Could you check a few things on this drawing? It's one solid part, dimensions in mm from its lowest x, y, z. A direction names the side the tool comes from. Give positions to 0.01 mm unless a question says otherwise; leave off trailing zeros. Loops run counter-clockwise (first coordinate to the right, second up) from the corner with the lowest first, then second, coordinate; pieces in that order, holes last. Notation, with made-up numbers: M 73.25,-15 L 101.25,-15 A24 ccw 101.25,-5 Z; hole C 29,65.5 d11. An arc over 180 degrees is marked long. Answer in a Markdown table with one row per item. Add a question column.
1. Which directions (+Z, -Z, +X, -X, +Y, -Y) give clear straight access to the entire face, cutting with the end or side of a thin tool? Please do the marked faces 1 and 2.
2. If we section it at D-D on x = 6: List the corners of the cut face in (y, z) for me, then the cut area to 3 significant figures.
3. Thinking about a two-plate mould opening in X: for the marked faces 3, 4, 5 and 6, which applies, released by +X, released by -X, zero draft, split by the parting line, or undercut?
4. If we section it at C-C on z = 3: List the corners of the cut face in (x, y) for me.
5. I need wall thicknesses on line 1 along Y through (x, z) = (34, 1.7); line 2 along Y through (x, z) = (34, 3.3); line 3 along X through (y, z) = (6.75, 5). Which ranges of each line are inside material? Lowest first, please. Write a range as from..to.
6. If we section it at B-B on y = 5: List the corners of the cut face in (x, z) for me.
7. I'm going to push flat-ended pins straight in: pin 1 Ø1.8 at (x, z) = (20.5, 4) entering from -Y; pin 2 Ø2.5 at (x, y) = (6, 5) entering from -Z; pin 3 Ø1.8 at (x, y) = (7, 6) entering from +Z; pin 4 Ø1.5 at (x, z) = (26, 3) entering from +Y. Where does each tip first touch, or does it pass through?
8. If we section it at A-A on x = 14: List the corners of the cut face in (y, z) for me.
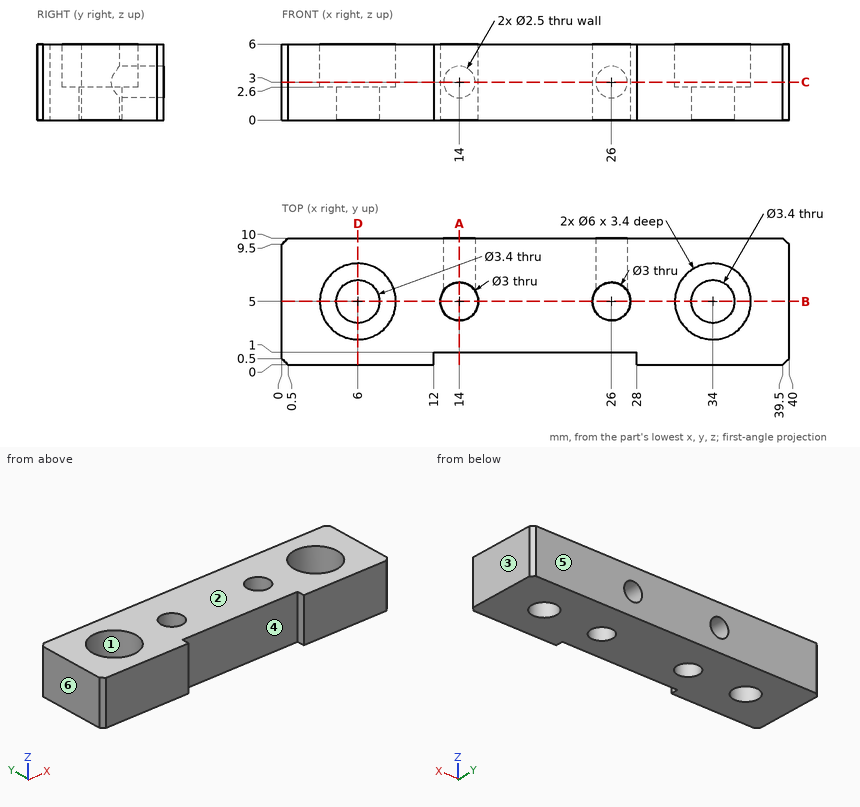
Results:
| question | item | result |
|---|---|---|
| 1 | face 1 | +Z |
| 1 | face 2 | +Z, +X, -X, +Y, -Y |
| 2 | outline | M 0,0 L 3.3,0 L 3.3,2.6 L 2,2.6 L 2,6 L 0,6 Z; M 6.7,0 L 10,0 L 10,6 L 8,6 L 8,2.6 L 6.7,2.6 Z |
| 2 | area | 30.8 mm2 |
| 3 | face 3 | released by +X |
| 3 | face 4 | undercut |
| 3 | face 5 | zero draft |
| 3 | face 6 | released by -X |
| 4 | outline | M 0,0.5 L 0.5,0 L 12,0 L 12,1 L 28,1 L 28,0 L 39.5,0 L 40,0.5 L 40,9.5 L 39.5,10 L 27.25,10 L 27.25,5.83 A1.5 cw long 24.75,5.83 L 24.75,10 L 15.25,10 L 15.25,5.83 A1.5 cw long 12.75,5.83 L 12.75,10 L 0.5,10 L 0,9.5 Z; hole C 6,5 d6; hole C 34,5 d6 |
| 5 | line 1 | 0..3.3, 6.7..10 |
| 5 | line 2 | 0..2, 8..10 |
| 5 | line 3 | 0..3.56, 8.44..31.56, 36.44..40 |
| 6 | outline | M 0,0 L 4.3,0 L 4.3,2.6 L 3,2.6 L 3,6 L 0,6 Z; M 7.7,0 L 12.5,0 L 12.5,6 L 9,6 L 9,2.6 L 7.7,2.6 Z; M 15.5,0 L 24.5,0 L 24.5,6 L 15.5,6 Z; M 27.5,0 L 32.3,0 L 32.3,2.6 L 31,2.6 L 31,6 L 27.5,6 Z; M 35.7,0 L 40,0 L 40,6 L 37,6 L 37,2.6 L 35.7,2.6 Z |
| 7 | pin 1 | y = 1 |
| 7 | pin 2 | through |
| 7 | pin 3 | z = 2.6 |
| 7 | pin 4 | y = 3.7 |
| 8 | outline | M 1,0 L 3.5,0 L 3.5,6 L 1,6 Z; M 6.5,0 L 10,0 L 10,1.75 L 6.5,1.75 Z; M 6.5,4.25 L 10,4.25 L 10,6 L 6.5,6 Z |
